from build123d import *

# Parameters (mm, degrees)
BASE_PLATE_SKETCH_R      = 9
BASE_PLATE_SKETCH_R_2    = 6
BASE_PLATE_SKETCH_R_3    = 4
BASE_PLATE_DEPTH         = 8
UPRIGHT_WEB_DEPTH        = 98
WEB_ANGLED_TRIM_SKETCH_R = 4
WEB_ANGLED_TRIM_DEPTH    = 98
PIVOT_LUG_SKETCH_R       = 6
PIVOT_LUG_DEPTH          = 6
LUG_CUT_SKETCH_R         = 6
LUG_CUT_DEPTH            = 16


with BuildPart() as part:
    # Base Plate Sketch → Base Plate (new body)
    with BuildSketch(Plane(origin=(0, 0, 0), x_dir=(1, 0, 0), z_dir=(0, 1, 0))):
        with BuildLine():
            Line((82, 32.334641746), (22.899881176, 32.334641746))
            ThreePointArc((22.899881176, 32.334641746), (14.88590337, 33.106300041), (7.166404253, 35.392919854))
            Line((7.166404253, 35.392919854), (-45.003147253, 56.470786852))
            ThreePointArc((-45.003147253, 56.470786852), (-54.304086029, 53.978607818), (-54.472135955, 44.351033997))
            Line((-54.472135955, 44.351033997), (-14.562305899, -10.580134541))
            ThreePointArc((-14.562305899, -10.580134541), (-5.562305899, -17.119017293), (5.562305899, -17.119017293))
            Line((5.562305899, -17.119017293), (85.708203932, 8.92196355))
            ThreePointArc((85.708203932, 8.92196355), (93.852260087, 22.211855326), (82, 32.334641746))
        make_face()
        with Locations(Location((0, 0, 0), (0, 0, 270))):
            Circle(BASE_PLATE_SKETCH_R, mode=Mode.SUBTRACT)
        with Locations(Location((82, 20.334641746, 0), (0, 0, 270))):
            Circle(BASE_PLATE_SKETCH_R_2, mode=Mode.SUBTRACT)
        with Locations(Location((-48, 49.053316016, 0), (0, 0, 270))):
            Circle(BASE_PLATE_SKETCH_R_3, mode=Mode.SUBTRACT)
    extrude(amount=BASE_PLATE_DEPTH)

    # Upright Web Sketch → Upright Web (add)
    with BuildSketch(Plane(origin=(0, 8, 0), x_dir=(1, 0, 0), z_dir=(0, 1, 0))):
        Polygon((-34.547004477, 16.926443267), (-10.806972302, 34.174586259), (-14.333683815, 39.028688225), (-38.07371599, 21.780545234), align=None)
        Polygon((37.898227453, -6.612439485), (28.456105239, 22.447424608), (34.162444337, 24.301526574), (43.604566551, -4.758337518), align=None)
    extrude(amount=UPRIGHT_WEB_DEPTH)

    # Web Angled Trim Sketch → Web Angled Trim (cut)
    with BuildSketch(Plane(origin=(-23.511410092, 0, -32.360679775), x_dir=(-0.8090169943749421, 0, 0.5877852522924805), z_dir=(-0.5877852522924805, 0, -0.8090169943749422))):
        with Locations((10, 46)):
            Circle(WEB_ANGLED_TRIM_SKETCH_R)
        with BuildLine():
            Line((-8.464278756, 8), (2.27259339, 48.070552361))
            ThreePointArc((2.27259339, 48.070552361), (11.044209538, 53.931558891), (18, 46))
            Line((18, 46), (24.045319571, 43.356543138))
            Line((24.045319571, 43.356543138), (48.419235534, 110.549500658))
            Line((48.419235534, 110.549500658), (-18.279656122, 110.549500658))
            Line((-18.279656122, 110.549500658), (-16.138704045, 8))
            Line((-16.138704045, 8), (-8.464278756, 8))
        make_face()
    extrude(amount=-WEB_ANGLED_TRIM_DEPTH, mode=Mode.SUBTRACT)

    # Pivot Lug Sketch → Pivot Lug (add)
    with BuildSketch(Plane(origin=(38.042260652, 0, -12.360679775), x_dir=(-0.3090169943749489, 0, -0.9510565162951532), z_dir=(0.9510565162951532, 0, -0.3090169943749489))):
        with BuildLine():
            Line((14.770349605, 8), (5.737771209, 50.49494029))
            ThreePointArc((5.737771209, 50.49494029), (-7.254341559, 59.934262744), (-18, 48))
            Line((-18, 48), (-18, 8))
            Line((-18, 8), (14.770349605, 8))
        make_face()
        with Locations((-6, 48)):
            Circle(PIVOT_LUG_SKETCH_R, mode=Mode.SUBTRACT)
    extrude(amount=-PIVOT_LUG_DEPTH)

    # Lug Cut Sketch → Lug Cut (cut)
    with BuildSketch(Plane(origin=(38.042260652, 0, -12.360679775), x_dir=(-0.3090169943749489, 0, -0.9510565162951532), z_dir=(0.9510565162951532, 0, -0.3090169943749489))):
        with Locations((-6, 48)):
            Circle(LUG_CUT_SKETCH_R)
        with BuildLine():
            Line((12.555349334, 18.420756966), (5.737771209, 50.49494029))
            ThreePointArc((5.737771209, 50.49494029), (-7.254341559, 59.934262744), (-18, 48))
            Line((-18, 48), (-46.797997281, 119.82194568))
            Line((-46.797997281, 119.82194568), (32.722077442, 114.455560269))
            Line((32.722077442, 114.455560269), (12.555349334, 18.420756966))
        make_face()
    extrude(amount=-LUG_CUT_DEPTH, mode=Mode.SUBTRACT)


solid = part.part
Can you work these out from the model? Positions are in its coordinate system, mm. A direction names the side the tool comes from. Round coordinates to 2 decimals unless told otherwise and drop trailing zeros. Write each loop counter-clockwise with the first axis right and the second up, starting at its lowest first coordinate (ties: lowest second). Pieces come first, ordered by that corner, then holes. Notation, with made-up numbers: (-37, 37) - (-17, 37) arc R15 cw to (-17, 66) - close; hole circle Ø7 at (31, 45). An arc over 180 degrees is marked (long way). Write each question's results on one line, items separated by ' | '. Start each with the question number.
1) Suppose I cut it at A-A (y = 38.5). List the corners of the cut face in (x, z) for me.
2) We'd pull the mould along X, two halves only. Please class faces 4 (the flat face through (53, 4, -32.335)), 5 (the cylindrical face through (14.997, 3.944, -33.085)), 6 (the cylindrical face through (-54.214, 3.944, -54.092)), 7 (the flat face through (-26.371, 25.567, -22.867)): released by +X, released by -X, zero draft, split by the parting line, or undercut.
3) Suppose I cut it at B-B (x = 0). List the corners of the cut face in (y, z) for me.
4) Which directions (+Z, -Z, +X, -X, +Y, -Y) give clear straight access to the entire face, cutting with the end or side of a thin tool? Please do faces 1 (the cylindrical face through (-5.71, 3.94, 17.07)), 2 (the flat face through (18, 8, -20)), 3 (the flat face through (-29.598, 25.567, -27.939)).
5) For pin 1 Ø4 at (x, y) = (-39.5, 34) entering from +Z; pin 2 Ø4 at (y, z) = (40.5, -19) entering from +X; pin 3 Ø10 at (x, z) = (7, -16.5) entering from -Y; pin 4 Ø22.5 at (x, z) = (13, -14) entering from +Y, each with a flat end and sliding along its axis, tell me the tip position at first contact or that it passes through.
6) Please list where these lines run through material, in increasing order: line 1 (Y direction, x = 49, z = -28.5); line 2 (X direction, y = 21, z = -21.5); line 3 (Y direction, x = -27.5, z = -25).
Here are the results:
1) outline: (-38.07, -21.78) - (-23.28, -32.53) - (-19.75, -27.68) - (-34.55, -16.93) - close; (29.77, -18.39) - (35.48, -20.24) - (43.6, 4.76) - (37.9, 6.61) - close
2) face 4: zero draft | face 5: released by +X | face 6: split by the parting line | face 7: undercut
3) outline: (0, -38.29) - (8, -38.29) - (8, -9) - (0, -9) - close; (0, 9) - (8, 9) - (8, 18) - (0, 18) - close
4) face 1: +Z, +Y, -Y | face 2: +Y | face 3: -Z, -X, +Y
5) pin 1: stops at z = -20.99 | pin 2: stops at x = 36.53 | pin 3: stops at y = 0 | pin 4: stops at y = 8
6) line 1: y = 0 to 8 | line 2: x = -37.87 to -28.25, 28.76 to 35.07 | line 3: y = 0 to 42.84, 49.16 to 53.62
